```python
from build123d import *

# Parameters (mm, degrees)
SKETCH_1_W                  = 60
SKETCH_1_H                  = 60
EXTRUDE_1_DEPTH             = 125
SKETCH_2_R                  = 25
EXTRUDE_2_DEPTH             = 3
SKETCH_3_R                  = 7
EXTRUDE_3_DEPTH             = 27
CUT_EXTRUDE_1_DEPTH         = 3
HOLE_WIZARD_M5_1_D          = 4.2
HOLE_WIZARD_M5_1_DEPTH      = 6
HOLE_WIZARD_M5_1_TIP        = 1.2618073
HOLE_WIZARD_4_5_4_5_1_D     = 5.5
HOLE_WIZARD_4_5_4_5_1_DEPTH = 10
HOLE_WIZARD_4_5_4_5_1_TIP   = 1.652366702
SKETCH_10_W                 = 9
SKETCH_10_H                 = 9
CUT_EXTRUDE_2_DEPTH         = 118.5
MIRROR_2_COPY_1_SKETCH_W    = 9
MIRROR_2_COPY_1_SKETCH_H    = 9
MIRROR_2_COPY_1_DEPTH       = 118.5
FILLET_1_R                  = 2


with BuildPart() as part:
    # 草图1 → 凸台-拉伸1 (new body)
    with BuildSketch(Plane.XY):
        Rectangle(SKETCH_1_W, SKETCH_1_H)
    extrude(amount=EXTRUDE_1_DEPTH)

    # 草图2 → 凸台-拉伸2 (add)
    with BuildSketch(Plane(origin=(0, 0, 0), x_dir=(-1, 0, 0), z_dir=(0, 0, -1))):
        with Locations(Location((0, 0, 0), (0, 0, 180))):
            Circle(SKETCH_2_R)
    extrude(amount=EXTRUDE_2_DEPTH)

    # 草图3 → 凸台-拉伸3 (add)
    with BuildSketch(Plane(origin=(0, 0, -3), x_dir=(-1, 0, 0), z_dir=(0, 0, -1))):
        Circle(SKETCH_3_R)
    extrude(amount=EXTRUDE_3_DEPTH)

    # 草图4 → 切除-拉伸1 (cut)
    with BuildSketch(Plane(origin=(0, 7, 0), x_dir=(1, 0, 0), z_dir=(0, 1, 0))):
        with BuildLine():
            Line((3, 30), (3, 7.5))
            ThreePointArc((3, 7.5), (0, 4.5), (-3, 7.5))
            Line((-3, 7.5), (-3, 30))
            ThreePointArc((-3, 30), (0, 33), (3, 30))
        make_face()
    extrude(amount=-CUT_EXTRUDE_1_DEPTH, mode=Mode.SUBTRACT)

    # M5 螺纹孔1
    with Locations(Plane(origin=(0, 0, -30), x_dir=(-1, 0, 0), z_dir=(0, 0, -1))):
        with Locations((0, 0)):
            Hole(HOLE_WIZARD_M5_1_D / 2, depth=HOLE_WIZARD_M5_1_DEPTH)
            with Locations((0, 0, -(HOLE_WIZARD_M5_1_DEPTH + HOLE_WIZARD_M5_1_TIP / 2))):  # 118° drill point
                Cone(0, HOLE_WIZARD_M5_1_D / 2, HOLE_WIZARD_M5_1_TIP, mode=Mode.SUBTRACT)

    # Ø4.5 (4.5) 直径孔1
    with Locations(Plane(origin=(0, 0, 0), x_dir=(-1, 0, 0), z_dir=(0, 0, -1))):
        with Locations((-24.748737342, 24.748737342), (24.748737342, 24.748737342), (24.748737342, -24.748737342), (-24.748737342, -24.748737342)):
            Hole(HOLE_WIZARD_4_5_4_5_1_D / 2, depth=HOLE_WIZARD_4_5_4_5_1_DEPTH)
            with Locations((0, 0, -(HOLE_WIZARD_4_5_4_5_1_DEPTH + HOLE_WIZARD_4_5_4_5_1_TIP / 2))):  # 118° drill point
                Cone(0, HOLE_WIZARD_4_5_4_5_1_D / 2, HOLE_WIZARD_4_5_4_5_1_TIP, mode=Mode.SUBTRACT)

    # 草图10 → 切除-拉伸2 (cut)
    with BuildSketch(Plane.XY.offset(125)):
        with Locations((-25.5, 25.5)):
            Rectangle(SKETCH_10_W, SKETCH_10_H)
    cut_extrude_2 = extrude(amount=-CUT_EXTRUDE_2_DEPTH, mode=Mode.SUBTRACT)

    # 镜向1: 切除-拉伸2 across plane
    add(cut_extrude_2.mirror(Plane(origin=(0, 0, 0), x_dir=(0, 0, 1), z_dir=(1, 0, 0))), mode=Mode.SUBTRACT)

    # 镜向2: 切除-拉伸2 across plane
    add(cut_extrude_2.mirror(Plane.ZX), mode=Mode.SUBTRACT)

    # 镜向2 copy 1 sketch → 镜向2 copy 1 (cut)
    with BuildSketch(Plane(origin=(0, 0, 125), x_dir=(-1, 0, 0), z_dir=(0, 0, 1))):
        with Locations((-25.5, 25.5)):
            Rectangle(MIRROR_2_COPY_1_SKETCH_W, MIRROR_2_COPY_1_SKETCH_H)
    extrude(amount=-MIRROR_2_COPY_1_DEPTH, mode=Mode.SUBTRACT)

    # 圆角1
    fillet_1_edges = [part.edges().sort_by_distance(p)[0] for p in [
        (-30, -30, 3.25),
        (-30, -21, 65.75),
        (-21, -21, 65.75),
        (-21, -30, 65.75),
        (-30, 30, 3.25),
        (-30, 21, 65.75),
        (-21, 30, 65.75),
        (-21, 21, 65.75),
        (30, 30, 3.25),
        (30, 21, 65.75),
        (21, 21, 65.75),
        (21, 30, 65.75),
        (30, -30, 3.25),
        (30, -21, 65.75),
        (21, -30, 65.75),
        (21, -21, 65.75),
    ]]
    fillet(fillet_1_edges, radius=FILLET_1_R)


solid = part.part
```
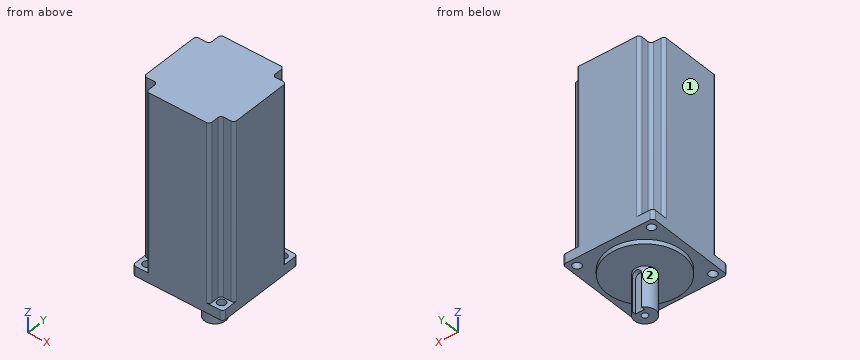
Model file for the job. Use its own axes, mm. Face numbers are marked on the shaded views. A direction names the side the tool comes from. Round coordinates to 2 decimals unless told otherwise and drop trailing zeros. Write each loop counter-clockwise with the first axis right and the second up, starting at its lowest first coordinate (ties: lowest second). Pieces come first, ordered by that corner, then holes. Notation, with made-up numbers: (53.5, 61.5) -> (86.5, 61.5) arc R24 cw to (86.5, 79.5) -> close; hole circle Ø10 at (-4, 2.5). An arc over 180 degrees is marked (long way). Answer as CSV lines item,"result".
1. Pin check, flat tips, straight feed: pin 1 Ø2.5 at (y, z) = (5.5, -20.5) entering from -X; pin 2 Ø1.5 at (y, z) = (26, 81.5) entering from +X; pin 3 Ø1.5 at (x, z) = (-25, 51.5) entering from -Y. Stop position of each tip, or through.
Resolved:
pin 1,"x = -5.56"
pin 2,"x = 21"
pin 3,"y = -21"
2. Slice it at D-D, the plane z = -15.5. List the corners of the cut face in (x, y).
Resolved:
outline,"(-3, 4) -> (-3, 6.32) arc R7 ccw (long way) to (3, 6.32) -> (3, 4) -> close"
3. Drill centre lines: line 1 (Z direction, x = -6, y = 8); line 2 (X direction, y = 25, z = 30.5); line 3 (Z direction, x = 22.5, y = -13). Where is each one in solid material? Low to high.
Resolved:
line 1,"-3 to 125"
line 2,"-21 to 21"
line 3,"0 to 125"
4. Slice it at B-B, the plane x = -10. List the corners of the cut face in (y, z).
Resolved:
outline,"(-30, 0) -> (-22.91, 0) -> (-22.91, -3) -> (22.91, -3) -> (22.91, 0) -> (30, 0) -> (30, 125) -> (-30, 125) -> close"
5. Slice it at A-A, the plane z = 91. List the corners of the cut face in (x, y).
Resolved:
outline,"(-30, -19) arc R2 ccw to (-28, -21) -> (-23, -21) arc R2 cw to (-21, -23) -> (-21, -28) arc R2 ccw to (-19, -30) -> (19, -30) arc R2 ccw to (21, -28) -> (21, -23) arc R2 cw to (23, -21) -> (28, -21) arc R2 ccw to (30, -19) -> (30, 19) arc R2 ccw to (28, 21) -> (23, 21) arc R2 cw to (21, 23) -> (21, 28) arc R2 ccw to (19, 30) -> (-19, 30) arc R2 ccw to (-21, 28) -> (-21, 23) arc R2 cw to (-23, 21) -> (-28, 21) arc R2 ccw to (-30, 19) -> close"
6. Tool access for the marked faces 1 and 2: list every direction of +Z, -Z, +X, -X, +Y, -Y with a clear straight run to the whole face (end or side of a thin tool).
Resolved:
face 1,"+Z, -Z, -X, +Y, -Y"
face 2,"-Z"
